Input: part model. Units: mm. Frame: model coordinates. Coordinates: 2 decimals unless noted, no trailing zeros. Write each loop counter-clockwise with the first axis right and the second up, starting at its lowest first coordinate (ties: lowest second). Pieces come first, ordered by that corner, then holes. Notation, with made-up numbers: (67, 37.25) - (101, 37.25) arc R31 cw to (101, 72.25) - close; hole circle Ø1 at (54, -18). An arc over 180 degrees is marked (long way). Use CSV: the item, a comma, the result in double quotes.
```python
from build123d import *

# Parameters (mm, degrees)
EXTRUDE1_DEPTH = 6


with BuildPart() as part:
    # Sketch1 → Extrude1 (new, symmetric)
    with BuildSketch(Plane(origin=(0, 0, 0), x_dir=(1, 0, 0), z_dir=(0, 1, 0))):
        Polygon((-15, -20), (-5, -20), (15, 10), (15, 20), (-15, 20), align=None)
    extrude(amount=EXTRUDE1_DEPTH, both=True)


solid = part.part
```
(1) Ray query, probe 1 along Z at (x, y) = (11.5, 4.25); probe 2 along X at (y, z) = (-2.5, 15.5); probe 3 along Z at (x, y) = (13.25, -3) (3 decimals). Return the intervals inside material, ascending. Write a range as from..to.
Check values:
probe 1,"-20..-4.75"
probe 2,"-15..-2"
probe 3,"-20..-7.375"
(2) Draft query along Z for faces 1 (the flat face through (5, 0, 5)), 2 (the flat face through (0, 0, -20)), 3 (the flat face through (-4, 6, -5)). Return one class per face: pulls with the +Z half, pulls with the -Z half, needs draft (parallel to the pull), parting line crosses it, or undercut.
Check values:
face 1,"pulls with the +Z half"
face 2,"pulls with the -Z half"
face 3,"needs draft"
(3) Cut plane B-B on x = -3.5. Return loops of the section in (y, z), and give its area (3 significant figures).
Check values:
outline,"(-6, -20) - (6, -20) - (6, 17.75) - (-6, 17.75) - close"
area,"453 mm^2"
(4) Cut plane A-A on y = 1.5. Return loops of the section in (x, z), and give its area (3 significant figures).
Check values:
outline,"(-15, -20) - (15, -20) - (15, -10) - (-5, 20) - (-15, 20) - close"
area,"900 mm^2"
(5) Cut plane C-C on z = 17. Return loops of the section in (x, y).
Check values:
outline,"(-15, -6) - (-3, -6) - (-3, 6) - (-15, 6) - close"
(6) Pin query (flat end, axial travel): pin 1 Ø6 at (y, z) = (4, -1) entering from +X; pin 2 Ø2 at (y, z) = (-4, 13) entering from +X. Return the tip coordinate at first contact, or that it passes through.
Check values:
pin 1,"x = 11"
pin 2,"x = 0.33"
